Verification items for the finished model (mm, model axes). Face numbers are marked on the shaded views. A direction names the side the tool comes from. Give positions to 0.01 mm unless a question says otherwise; leave off trailing zeros. Loops run counter-clockwise (first coordinate to the right, second up) from the corner with the lowest first, then second, coordinate; pieces in that order, holes last. Notation, with made-up numbers: (67.25, -35.75) -> (107.25, -35.75) arc R17 cw to (107.25, -8.75) -> close; hole circle Ø3 at (6, -16.5). An arc over 180 degrees is marked (long way). Answer in a Markdown table with one row per item. Add a question column.
Q1. Material ranges on probe 1 along Z at (x, y) = (22, 33.5); probe 2 along Y at (x, z) = (9.5, -14.5); probe 3 along Y at (x, z) = (-26.5, 19.5), recorded low to high.
Q2. Section check D-D on z = -0.5. Enter the section's corners in (x, y), and give its area (3 significant figures).
Q3. Gauge pin test, flat ends, axial feed: P1, Ø16, axis at x = 17.5, z = -0.5, coming from the +Y side; P2, Ø20, axis at x = 4, y = 42.5, coming from the +Z side; P3, Ø7.5, axis at x = 8, z = -14.5, coming from the +Y side. Record the tip position at first contact, or that the pin passes through.
Q4. Section check B-B on y = 9. Enter the section's corners in (x, z).
Q5. Section check A-A on z = -13.5. Enter the section's corners in (x, y).
Q6. Set-up check for the marked faces 1, 2, 3, 4 and 5: record each of +Z, -Z, +X, -X, +Y, -Y from which the full face is reachable in a straight line by a thin tool's end or side.
Q7. Section check C-C on x = -16. Enter the section's corners in (y, z), and give its area (3 significant figures).
Q8. Release check for a two-part mould opening along Y. For the marked faces 6, 7 and 8 record: pulls with the +Y half, pulls with the -Y half, needs draft (parallel to the pull), parting line crosses it, or undercut.
```python
from build123d import *

# Parameters (mm, degrees)
STEPPED_BLOCK_60MM_DEPTH             = 30
UNDERSIDE_DOVETAIL_GROOVE_REACH      = 70.007
UNDERSIDE_DOVETAIL_GROOVE_SKETCH_W   = 15
UNDERSIDE_DOVETAIL_GROOVE_SKETCH_H   = 15
UNDERSIDE_DOVETAIL_GROOVE_SKETCH_W_2 = 25
TOP_TIER_POCKET_30X20_REACH          = 84.006


with BuildPart() as part:
    # Stepped Block Profile Sketch → Stepped Block 60mm (new, symmetric)
    with BuildSketch(Plane(origin=(0, 0, 0), x_dir=(0, 0, -1), z_dir=(1, 0, 0))):
        Polygon((-25, 0), (25, 0), (25, 25), (10, 25), (10, 50), (-10, 50), (-10, 25), (-25, 25), align=None)
    extrude(amount=STEPPED_BLOCK_60MM_DEPTH, both=True)

    # Underside Dovetail Groove Sketch → Underside Dovetail Groove (cut, up to next)
    with BuildSketch(Plane.XY.offset(10), mode=Mode.PRIVATE) as underside_dovetail_groove_sk1:
        with Locations((-22.5, 42.5)):
            Rectangle(UNDERSIDE_DOVETAIL_GROOVE_SKETCH_W, UNDERSIDE_DOVETAIL_GROOVE_SKETCH_H)
    underside_dovetail_groove_tool1 = extrude(underside_dovetail_groove_sk1.sketch, amount=-UNDERSIDE_DOVETAIL_GROOVE_REACH, mode=Mode.PRIVATE) & part.part
    # Underside Dovetail Groove Sketch → Underside Dovetail Groove (cut, up to next)
    with BuildSketch(Plane.XY.offset(10), mode=Mode.PRIVATE) as underside_dovetail_groove_sk2:
        with Locations((17.5, 42.5)):
            Rectangle(UNDERSIDE_DOVETAIL_GROOVE_SKETCH_W_2, UNDERSIDE_DOVETAIL_GROOVE_SKETCH_H)
    underside_dovetail_groove_tool2 = extrude(underside_dovetail_groove_sk2.sketch, amount=-UNDERSIDE_DOVETAIL_GROOVE_REACH, mode=Mode.PRIVATE) & part.part
    add(underside_dovetail_groove_tool1.solids().sort_by_distance((-22.5, 42.5, 10))[0], mode=Mode.SUBTRACT)
    add(underside_dovetail_groove_tool2.solids().sort_by_distance((17.5, 42.5, 10))[0], mode=Mode.SUBTRACT)

    # Top Tier Pocket Sketch → Top Tier Pocket 30x20 (cut, up to next)
    with BuildSketch(Plane(origin=(30, 0, 0), x_dir=(0, 0, -1), z_dir=(1, 0, 0)), mode=Mode.PRIVATE) as top_tier_pocket_30x20_sk1:
        Polygon((-10, 0), (-15, 10), (15, 10), (10, 0), align=None)
    top_tier_pocket_30x20_tool1 = extrude(top_tier_pocket_30x20_sk1.sketch, amount=-TOP_TIER_POCKET_30X20_REACH, mode=Mode.PRIVATE) & part.part
    add(top_tier_pocket_30x20_tool1.solids().sort_by_distance((30, 5.333333, 0))[0], mode=Mode.SUBTRACT)


solid = part.part
```
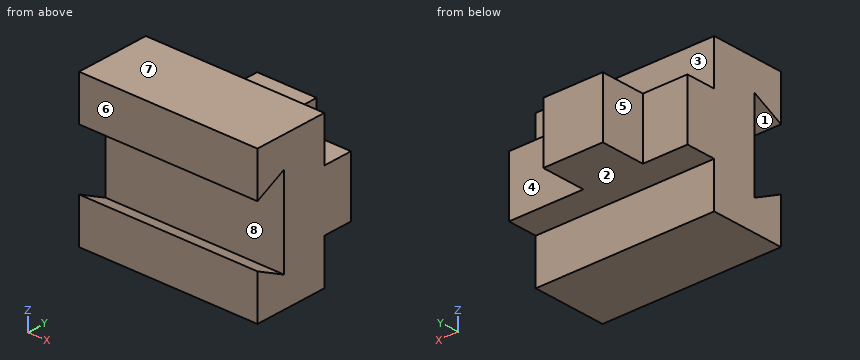
Taken from the geometry:
| question | item | result |
|---|---|---|
| 1 | probe 1 | z = -10 to 10 |
| 1 | probe 2 | y = 0 to 9, 10 to 25 |
| 1 | probe 3 | y = 0 to 25 |
| 2 | outline | (-30, 10) -> (30, 10) -> (30, 35) -> (5, 35) -> (5, 50) -> (-15, 50) -> (-15, 35) -> (-30, 35) -> close |
| 2 | area | 1,800 mm² |
| 3 | P1 | stops at y = 35 |
| 3 | P2 | stops at z = 10 |
| 3 | P3 | stops at y = 25 |
| 4 | outline | (-30, -25) -> (30, -25) -> (30, -14.5) -> (-30, -14.5) -> close; (-30, 14.5) -> (30, 14.5) -> (30, 25) -> (-30, 25) -> close |
| 5 | outline | (-30, 0) -> (30, 0) -> (30, 7) -> (-30, 7) -> close; (-30, 10) -> (30, 10) -> (30, 25) -> (-30, 25) -> close |
| 6 | face 1 | +X, -X |
| 6 | face 2 | -Z, +X, -X, +Y |
| 6 | face 3 | +Z, +X, -X, +Y |
| 6 | face 4 | +Z, -Z, +X, +Y |
| 6 | face 5 | +Z, -Z, -X, +Y |
| 7 | outline | (0, -25) -> (25, -25) -> (25, -10) -> (35, -10) -> (35, 10) -> (25, 10) -> (25, 25) -> (0, 25) -> (0, 10) -> (10, 15) -> (10, -15) -> (0, -10) -> close |
| 7 | area | 1,200 mm² |
| 8 | face 6 | pulls with the -Y half |
| 8 | face 7 | needs draft |
| 8 | face 8 | undercut |
